Here's the drawing with two shaded views (mm, measured from the low corner). I have some questions. Give positions to 0.01 mm unless a question says otherwise; leave off trailing zeros. Write each loop counter-clockwise with the first axis right and the second up, starting at its lowest first coordinate (ties: lowest second). Pieces come first, ordered by that corner, then holes. Notation, with made-up numbers: (3.25, 81) -> (17.25, 81) arc R22 cw to (17.25, 96) -> close; hole circle Ø10 at (-30.75, -31). An arc over 180 degrees is marked (long way). One line per item, written item: value.
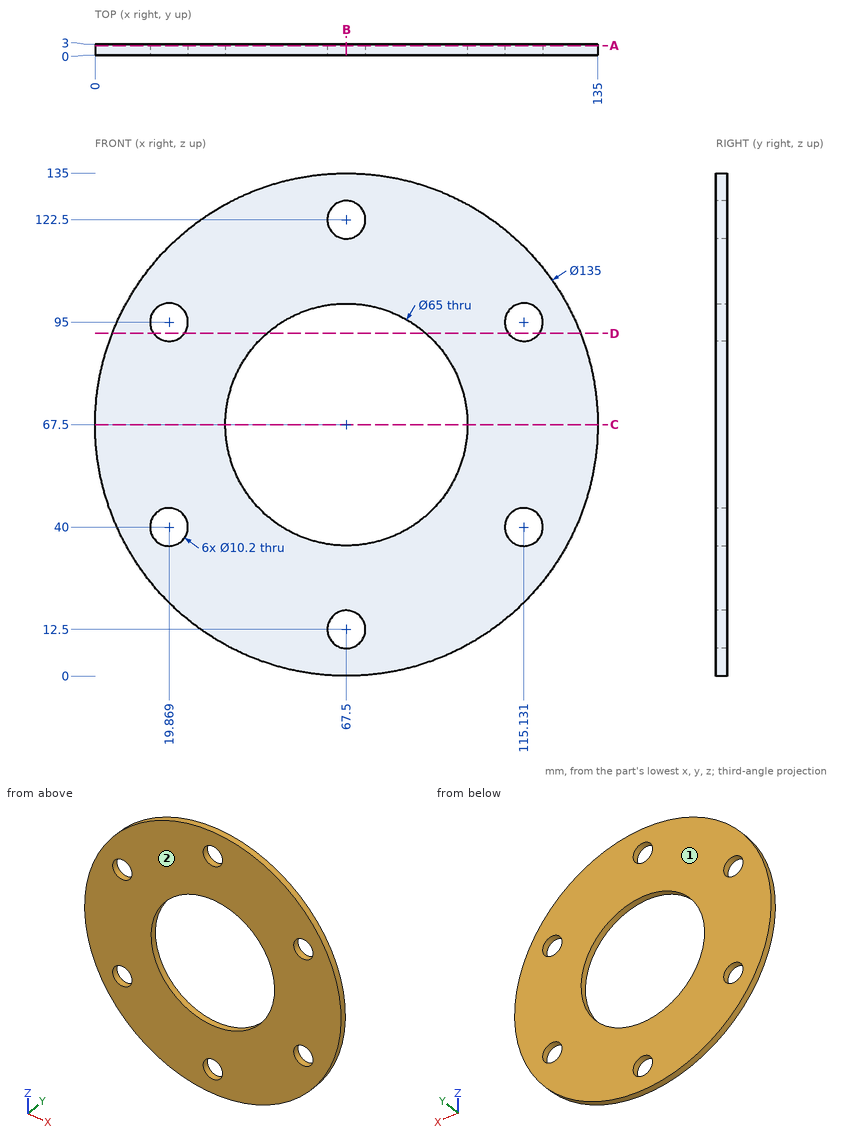
1) I need wall thicknesses on L1, parallel to X at y = 0.7, z = 95 (1 decimal); L2, parallel to X at y = 1.65, z = 67.5; L3, parallel to X at y = 1, z = 97.5 (1 decimal). Which ranges of each line are inside material? Lowest first, please.
Answer list:
L1: x = 5.9 to 14.8, 25 to 50.2, 84.8 to 110, 120.2 to 129.1
L2: x = 0 to 35, 100 to 135
L3: x = 7 to 15.4, 24.3 to 55, 80 to 110.7, 119.6 to 128
2) If we section it at D-D (z = 92): Write out the boundary of the cut face in (x, y) (1 decimal), and give its area (3 significant figures).
Answer list:
outline: (4.6, 0) -> (15.7, 0) -> (15.7, 3) -> (4.6, 3) -> close; (24, 0) -> (46.1, 0) -> (46.1, 3) -> (24, 3) -> close; (88.9, 0) -> (111, 0) -> (111, 3) -> (88.9, 3) -> close; (119.3, 0) -> (130.4, 0) -> (130.4, 3) -> (119.3, 3) -> close
area: 200 mm^2
3) Will this pin go through, and if not, where does the flat tip stop? pin 1 (13.5 mm diameter, centred on x = 67.5, z = 12.5, fed in from +Y).
Answer list:
pin 1: stops at y = 3
4) If we section it at C-C (z = 67.5): Write out the boundary of the cut face in (x, y), and give its area (3 significant figures).
Answer list:
outline: (0, 0) -> (35, 0) -> (35, 3) -> (0, 3) -> close; (100, 0) -> (135, 0) -> (135, 3) -> (100, 3) -> close
area: 210 mm^2
5) If we section it at B-B (x = 67.5): Write out the boundary of the cut face in (y, z).
Answer list:
outline: (0, 0) -> (3, 0) -> (3, 7.4) -> (0, 7.4) -> close; (0, 17.6) -> (3, 17.6) -> (3, 35) -> (0, 35) -> close; (0, 100) -> (3, 100) -> (3, 117.4) -> (0, 117.4) -> close; (0, 127.6) -> (3, 127.6) -> (3, 135) -> (0, 135) -> close
6) If we section it at A-A (y = 2.55): Write out the boundary of the cut face in (x, z).
Answer list:
outline: circle Ø135 at (67.5, 67.5); hole circle Ø10.2 at (19.87, 40); hole circle Ø10.2 at (19.87, 95); hole circle Ø65 at (67.5, 67.5); hole circle Ø10.2 at (67.5, 12.5); hole circle Ø10.2 at (67.5, 122.5); hole circle Ø10.2 at (115.13, 40); hole circle Ø10.2 at (115.13, 95)
7) We'd pull the mould along Y, two halves only. Please class the marked faces 1 and 2: released by +Y, released by -Y, zero draft, split by the parting line, or undercut.
Answer list:
face 1: released by +Y
face 2: released by -Y
